Design review of the part built by this model. Coordinates are the model's own, in mm. Face numbers are marked on the shaded views. A direction names the side the tool comes from. Round coordinates to 2 decimals unless told otherwise and drop trailing zeros. Loops run counter-clockwise (first coordinate to the right, second up) from the corner with the lowest first, then second, coordinate; pieces in that order, holes last. Notation, with made-up numbers: (5.25, 66.25) - (14.25, 66.25) arc R16 ccw to (14.25, 75.25) - close; hole circle Ø11 at (47.25, 36). An arc over 180 degrees is marked (long way). Return JSON: item names as keys, results as strings. Group by question number.
(1) For the marked faces 4, 5 and 6, list the 3-axis set-ups (+Z, -Z, +X, -X, +Y, -Y) from which the entire face can be reached by the end or side of a thin tool; tool diameter is ignored.
(2) Wall thickness on L1, parallel to Y at x = 10, z = 6; L2, parallel to Z at x = 75, y = 35.5; L3, parallel to X at y = 7, z = 49: over which ranges is each line inside the solid? List them lowest first. Write a range as [from, to].
(3) We need section B-B, the plane y = 25. Write out the cut boundary in (x, z), and give its area (3 significant figures).
(4) We need section A-A, the plane x = 44. Write out the cut boundary in (y, z), and give its area (3 significant figures).
(5) We need section C-C, the plane z = 6. Write out the cut boundary in (x, y), and give its area (3 significant figures).
(6) Clearance check with flat-ended pins moving along their axes: pin 1 (11 mm diameter, centred on y = 14.5, z = 45, fed in from +X); pin 2 (10.5 mm diameter, centred on x = 83, y = 23.5, fed in from +Z); pin 3 (1 mm diameter, centred on y = 18.5, z = 49, fed in from -X). State where each tip first meets the part, or that it passes through.
(7) We need section D-D, the plane z = 48.5. Write out the cut boundary in (x, y).
(8) The part is to be moulded in two halves that separate along X. For the marked faces 1, 2 and 3, say which applies: pulls with the +X half, pulls with the -X half, needs draft (parallel to the pull), parting line crosses it, or undercut.
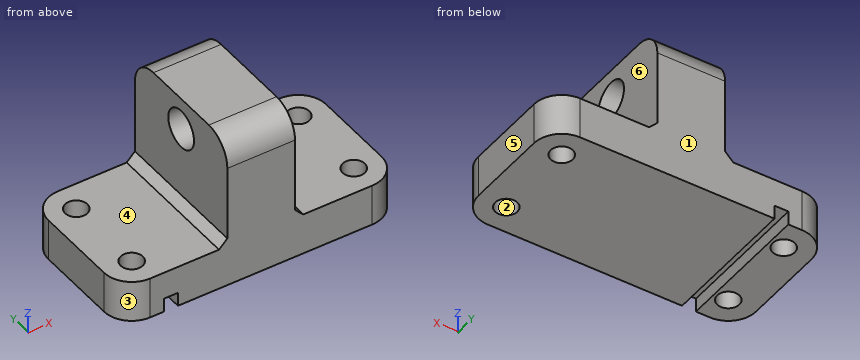
from build123d import *

# Parameters (mm, degrees)
BASE_PLATE_DEPTH              = 15
KNUCKLE_BLOCK_DEPTH           = 100
KNUCKLE_RELIEF_CUT_A_DEPTH    = 37.8
KNUCKLE_START                 = -37.8
KNUCKLE_RELIEF_CUT_B_DEPTH    = 37.8
PLATE_MOUNTING_HOLES_SKETCH_W = 5
PLATE_MOUNTING_HOLES_SKETCH_H = 5
PLATE_MOUNTING_HOLES_DEPTH    = 50
HINGE_PIN_HOLE_SKETCH_R       = 6.957950298
HINGE_PIN_HOLE_DEPTH          = 50
UPPER_MOUNTING_HOLES_SKETCH_R = 4
UPPER_MOUNTING_HOLES_DEPTH    = 50
KNUCKLE_CHAMFER_A_3X45_SIZE   = 3
KNUCKLE_CHAMFER_B_3X45_SIZE   = 3


with BuildPart() as part:
    # Base Plate Sketch → Base Plate (new body)
    with BuildSketch(Plane.XY):
        with BuildLine():
            Line((10, 0), (90, 0))
            ThreePointArc((90, 0), (97.071067812, 2.928932188), (100, 10))
            Line((100, 10), (100, 40))
            ThreePointArc((100, 40), (97.071067812, 47.071067812), (90, 50))
            Line((90, 50), (10, 50))
            ThreePointArc((10, 50), (2.928932188, 47.071067812), (0, 40))
            Line((0, 40), (0, 10))
            ThreePointArc((0, 10), (2.928932188, 2.928932188), (10, 0))
        make_face()
    extrude(amount=BASE_PLATE_DEPTH)

    # Knuckle Block Sketch → Knuckle Block (add)
    with BuildSketch(Plane(origin=(100, 0, 0), x_dir=(0, 0, -1), z_dir=(1, 0, 0))):
        with BuildLine():
            Line((-15, 50), (-45, 50))
            ThreePointArc((-45, 50), (-52.071067812, 47.071067812), (-55, 40))
            Line((-55, 40), (-55, 10))
            ThreePointArc((-55, 10), (-52.071067812, 2.928932188), (-45, 0))
            Line((-45, 0), (-15, 0))
            Line((-15, 0), (-15, 50))
        make_face()
    extrude(amount=-KNUCKLE_BLOCK_DEPTH)

    # Knuckle Relief Cut A Sketch → Knuckle Relief Cut A (cut)
    with BuildSketch(Plane(origin=(100, 0, 0), x_dir=(0, 0, -1), z_dir=(1, 0, 0))):
        with BuildLine():
            Line((-15, 40), (-15, 50))
            Line((-15, 50), (-45, 50))
            ThreePointArc((-45, 50), (-52.071067812, 47.071067812), (-55, 40))
            Line((-55, 40), (-55, 10))
            ThreePointArc((-55, 10), (-52.071067812, 2.928932188), (-45, 0))
            Line((-45, 0), (-15, 0))
            Line((-15, 0), (-15, 40))
        make_face()
    extrude(amount=-KNUCKLE_RELIEF_CUT_A_DEPTH, mode=Mode.SUBTRACT)

    # Knuckle Relief Cut B Sketch → Knuckle Relief Cut B (cut)
    with BuildSketch(Plane.ZY.offset(KNUCKLE_START)):
        with BuildLine():
            Line((15, 50), (45, 50))
            ThreePointArc((45, 50), (52.071067812, 47.071067812), (55, 40))
            Line((55, 40), (55, 10))
            ThreePointArc((55, 10), (52.071067812, 2.928932188), (45, 0))
            Line((45, 0), (15, 0))
            Line((15, 0), (15, 50))
        make_face()
    extrude(amount=KNUCKLE_RELIEF_CUT_B_DEPTH, mode=Mode.SUBTRACT)

    # Plate Mounting Holes Sketch → Plate Mounting Holes (cut)
    with BuildSketch(Plane.XZ):
        with Locations((17.5, 2.5)):
            Rectangle(PLATE_MOUNTING_HOLES_SKETCH_W, PLATE_MOUNTING_HOLES_SKETCH_H)
    extrude(amount=-PLATE_MOUNTING_HOLES_DEPTH, mode=Mode.SUBTRACT)

    # Hinge Pin Hole Sketch → Hinge Pin Hole (cut)
    with BuildSketch(Plane(origin=(62.2, 0, 0), x_dir=(0, 0, -1), z_dir=(1, 0, 0))):
        with Locations((-43.415970908, 25)):
            Circle(HINGE_PIN_HOLE_SKETCH_R)
    extrude(amount=-HINGE_PIN_HOLE_DEPTH, mode=Mode.SUBTRACT)

    # Upper Mounting Holes Sketch → Upper Mounting Holes (cut)
    with BuildSketch(Plane.XY.offset(15)):
        with Locations((90, 40)):
            Circle(UPPER_MOUNTING_HOLES_SKETCH_R)
        with Locations((90, 10)):
            Circle(UPPER_MOUNTING_HOLES_SKETCH_R)
        with Locations((10, 40)):
            Circle(UPPER_MOUNTING_HOLES_SKETCH_R)
        with Locations((10, 10)):
            Circle(UPPER_MOUNTING_HOLES_SKETCH_R)
    extrude(amount=-UPPER_MOUNTING_HOLES_DEPTH, mode=Mode.SUBTRACT)

    # Knuckle Chamfer A 3x45
    knuckle_chamfer_a_3x45_edges = [part.edges().sort_by_distance(p)[0] for p in [
        (62.2, 25, 15),
    ]]
    chamfer(knuckle_chamfer_a_3x45_edges, length=KNUCKLE_CHAMFER_A_3X45_SIZE)

    # Knuckle Chamfer B 3x45
    knuckle_chamfer_b_3x45_edges = [part.edges().sort_by_distance(p)[0] for p in [
        (37.8, 25, 15),
    ]]
    chamfer(knuckle_chamfer_b_3x45_edges, length=KNUCKLE_CHAMFER_B_3X45_SIZE)


solid = part.part
Solutions:
{
 "1": {"face 4": "+Z, -X, +Y, -Y", "face 5": "+Z, -Z, +X, +Y, -Y", "face 6": "+Z, +X, +Y, -Y"},
 "2": {"L1": "[0, 6], [14, 36], [44, 50]", "L2": "[0, 15]", "L3": "[37.8, 62.2]"},
 "3": {"outline": "(0, 0) - (15, 0) - (15, 5) - (20, 5) - (20, 0) - (100, 0) - (100, 15) - (65.2, 15) - (62.2, 18) - (62.2, 36.46) - (37.8, 36.46) - (37.8, 18) - (34.8, 15) - (0, 15) - close; (37.8, 50.37) - (62.2, 50.37) - (62.2, 55) - (37.8, 55) - close", "area": "2,120 mm^2"},
 "4": {"outline": "(0, 0) - (50, 0) - (50, 45) arc R10 ccw to (40, 55) - (10, 55) arc R10 ccw to (0, 45) - close; hole circle Ø13.92 at (25, 43.42)", "area": "2,550 mm^2"},
 "5": {"outline": "(0, 10) arc R10 ccw to (10, 0) - (90, 0) arc R10 ccw to (100, 10) - (100, 40) arc R10 ccw to (90, 50) - (10, 50) arc R10 ccw to (0, 40) - close; hole circle Ø8 at (10, 10); hole circle Ø8 at (10, 40); hole circle Ø8 at (90, 10); hole circle Ø8 at (90, 40)", "area": "4,710 mm^2"},
 "6": {"pin 1": "x = 62.2", "pin 2": "z = 15", "pin 3": "x = 37.8"},
 "7": {"outline": "(37.8, 0.63) - (62.2, 0.63) - (62.2, 20.25) - (37.8, 20.25) - close; (37.8, 29.75) - (62.2, 29.75) - (62.2, 49.37) - (37.8, 49.37) - close"},
 "8": {"face 1": "needs draft", "face 2": "undercut", "face 3": "pulls with the -X half"}
}
